```python
from build123d import *

# Parameters (mm, degrees)
SKETCH1_W              = 120
SKETCH1_H              = 505
BOSS_EXTRUDE1_DEPTH    = 10
M12_TAPPED_HOLE1_D     = 10.2
M12_TAPPED_HOLE1_DEPTH = 29.25
M12_TAPPED_HOLE1_TIP   = 3.064389157


with BuildPart() as part:
    # Sketch1 → Boss-Extrude1 (new body)
    with BuildSketch(Plane.XY):
        Rectangle(SKETCH1_W, SKETCH1_H)
    extrude(amount=BOSS_EXTRUDE1_DEPTH)

    # M12 Tapped Hole1
    with Locations(Plane.XY.offset(10)):
        with Locations((-32.5, 217.5), (32.5, 217.5), (32.5, -217.5), (-32.5, -217.5)):
            Hole(M12_TAPPED_HOLE1_D / 2, depth=M12_TAPPED_HOLE1_DEPTH)
            with Locations((0, 0, -(M12_TAPPED_HOLE1_DEPTH + M12_TAPPED_HOLE1_TIP / 2))):  # 118° drill point
                Cone(0, M12_TAPPED_HOLE1_D / 2, M12_TAPPED_HOLE1_TIP, mode=Mode.SUBTRACT)


solid = part.part
```
Verification items for the finished model (mm, model axes). Give positions to 0.01 mm unless a question says otherwise; leave off trailing zeros. Order: outer loops, then holes, each group sorted by start corner. A loop starts at its lowest first (then second) coordinate and runs counter-clockwise, first axis right, second up. Notation, with made-up numbers: M 85.25,37.5 L 124.25,37.5 A21 cw 124.25,60.5 Z; hole C 44,56 d6. An arc over 180 degrees is marked long. Return JSON: item names as keys, results as strings. Group by question number.
1) Section check A-A on x = 32.5. Record the cut outline in (y, z).
2) Mould release check, pull along Y, two halves, no side actions. Record for faces 1 (the face through (-1, 252.5, 5)), 2 (the face through (60, -4, 5)), 3 (the face through (-31.836, 222.557, 4.93)): pulls with the +Y half, pulls with the -Y half, needs draft (parallel to the pull), parting line crosses it, or undercut.
3) Section check B-B on y = -217.5. Record the cut outline in (x, z).
4) Scan lines: line 1 (Y direction, x = -32.5, z = 7.5); line 2 (X direction, y = -221, z = 8). Record each from-to range of solid material in increasing order.
5) Go/stop test with flat-tipped pins: pin 1 Ø16.5 at (x, y) = (-32.5, -217.5) entering from -Z; pin 2 Ø6 at (x, y) = (-32.5, 217.5) entering from -Z. Record where each tip stops, or that it passes through.
Answer block:
{
 "1": {"outline": "M -252.5,0 L -222.6,0 L -222.6,10 L -252.5,10 Z; M -212.4,0 L 212.4,0 L 212.4,10 L -212.4,10 Z; M 222.6,0 L 252.5,0 L 252.5,10 L 222.6,10 Z"},
 "2": {"face 1": "pulls with the +Y half", "face 2": "needs draft", "face 3": "undercut"},
 "3": {"outline": "M -60,0 L -37.6,0 L -37.6,10 L -60,10 Z; M -27.4,0 L 27.4,0 L 27.4,10 L -27.4,10 Z; M 37.6,0 L 60,0 L 60,10 L 37.6,10 Z"},
 "4": {"line 1": "y = -252.5 to -222.6, -212.4 to 212.4, 222.6 to 252.5", "line 2": "x = -60 to -36.21, -28.79 to 28.79, 36.21 to 60"},
 "5": {"pin 1": "stops at z = 0", "pin 2": "passes through"}
}
